Geometry check sheet. Reference: the model listing, model coordinates, mm. Face numbers are marked on the shaded views. Give positions to 0.01 mm unless a question says otherwise; leave off trailing zeros. Write each loop counter-clockwise with the first axis right and the second up, starting at its lowest first coordinate (ties: lowest second). Pieces come first, ordered by that corner, then holes. Notation, with made-up numbers: M -28.75,38 L 23.25,38 A34 ccw 23.25,74 Z; hole C 26.5,-10.5 d3. An arc over 180 degrees is marked long. Use one line per item in the form item = value. Start each with the question number.
```python
from build123d import *

# Parameters (mm, degrees)
EXTRUDE_1_DEPTH    = 17.5
CHAMFER_1_SIZE     = 2
HOLE_WIZARD_M5_1_D = 4.2


with BuildPart() as part:
    # 草图1 → 凸台-拉伸1 (new, symmetric)
    with BuildSketch(Plane(origin=(0, 0, 0), x_dir=(1, 0, 0), z_dir=(0, 1, 0))):
        with BuildLine():
            Line((7.5, 9.949874371), (7.5, 20))
            Line((7.5, 20), (-7.5, 20))
            Line((-7.5, 20), (-7.5, -20))
            Line((-7.5, -20), (7.5, -20))
            Line((7.5, -20), (7.5, -9.949874371))
            ThreePointArc((7.5, -9.949874371), (-1.5, 0), (7.5, 9.949874371))
        make_face()
    extrude(amount=EXTRUDE_1_DEPTH, both=True)

    # 倒角1
    chamfer_1_edges = [part.edges().sort_by_distance(p)[0] for p in [
        (0, 17.5, 20),
        (0, 17.5, -20),
        (0, -17.5, 20),
        (0, -17.5, -20),
    ]]
    chamfer(chamfer_1_edges, length=CHAMFER_1_SIZE)

    # M5 螺纹孔1 (through all)
    with Locations(Plane(origin=(7.5, 0, 0), x_dir=(0, 0, -1), z_dir=(1, 0, 0))):
        with Locations((-14, 10), (14, 10), (14, -10), (-14, -10)):
            Hole(HOLE_WIZARD_M5_1_D / 2)


solid = part.part
```
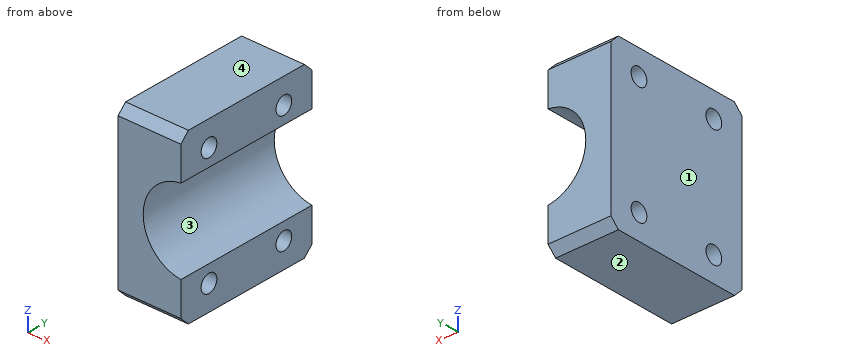
(1) Sectioned sample at C-C, the plane y = -10. Record the boundary of the cut face in (x, z).
(2) Sectioned sample at B-B, the plane x = 3. Record the boundary of the cut face in (y, z), plus the area to 3 significant figures.
(3) Thickness scan on probe 1 along Y at (x, z) = (4, 14); probe 2 along Z at (x, y) = (-5, 9); probe 3 along Z at (x, y) = (5.5, -11). Record the ranges inside material, lowest first. Write a range as [from, to].
(4) Draft check along Z on the marked faces 1, 2, 3 and 4. Enter one of: released by +Z, released by -Z, zero draft, split by the parting line, or undercut.
(5) Depth check by flat-ended pin: pin 1 (1 mm diameter, centred on y = 0.5, z = -8, fed in from +X); pin 2 (5 mm diameter, centred on y = -9.5, z = -14, fed in from -X). Enter the tip coordinate at first touch or a pass-through.
(6) Sectioned sample at D-D, the plane y = -6. Record the boundary of the cut face in (x, z), plus the area to 3 significant figures.
(7) Sectioned sample at A-A, the plane z = 14. Record the boundary of the cut face in (x, y), plus the area to 3 significant figures.
Numbers:
q1.outline = M -7.5,-20 L 7.5,-20 L 7.5,-16.1 L -7.5,-16.1 Z; M -7.5,-11.9 L 7.5,-11.9 L 7.5,-9.95 A10 cw 7.5,9.95 L 7.5,11.9 L -7.5,11.9 Z; M -7.5,16.1 L 7.5,16.1 L 7.5,20 L -7.5,20 Z
q2.outline = M -17.5,-18 L -15.5,-20 L 15.5,-20 L 17.5,-18 L 17.5,-8.35 L -17.5,-8.35 Z; M -17.5,8.35 L 17.5,8.35 L 17.5,18 L 15.5,20 L -15.5,20 L -17.5,18 Z; hole C -10,-14 d4.2; hole C -10,14 d4.2; hole C 10,-14 d4.2; hole C 10,14 d4.2
q2.area = 752 mm2
q3.probe_1 = [-17.5, -12.1], [-7.9, 7.9], [12.1, 17.5]
q3.probe_2 = [-20, -15.85], [-12.15, 12.15], [15.85, 20]
q3.probe_3 = [-20, -15.85], [-12.15, -9.54], [9.54, 12.15], [15.85, 20]
q4.face_1 = zero draft
q4.face_2 = released by -Z
q4.face_3 = undercut
q4.face_4 = released by +Z
q5.pin_1 = 3.23
q5.pin_2 = -7.5
q6.outline = M -7.5,-20 L 7.5,-20 L 7.5,-9.95 A10 cw 7.5,9.95 L 7.5,20 L -7.5,20 Z
q6.area = 463 mm2
q7.outline = M -7.5,-17.5 L 7.5,-17.5 L 7.5,-12.1 L -7.5,-12.1 Z; M -7.5,-7.9 L 7.5,-7.9 L 7.5,7.9 L -7.5,7.9 Z; M -7.5,12.1 L 7.5,12.1 L 7.5,17.5 L -7.5,17.5 Z
q7.area = 399 mm2
